```python
from build123d import *

# Parameters (mm, degrees)
BOSS_EXTRUDE1_DEPTH = 150
SKETCH2_R           = 1.500003704
SKETCH2_R_2         = 1.500002005
SKETCH2_R_3         = 1.500336032
SKETCH2_R_4         = 1.499979566
CUT_EXTRUDE1_DEPTH  = 5
SKETCH7_W           = 12.7
SKETCH7_H           = 16.8
CUT_EXTRUDE2_DEPTH  = 13
SKETCH8_W           = 16.8
SKETCH8_H           = 12.7
CUT_EXTRUDE3_DEPTH  = 13
SKETCH9_W           = 12.7
SKETCH9_H           = 16.8
CUT_EXTRUDE4_DEPTH  = 13
SKETCH10_W          = 18.7
SKETCH10_H          = 22.8
CUT_EXTRUDE5_DEPTH  = 2
FILLET1_R           = 2
SKETCH12_W          = 22.8
SKETCH12_H          = 18.7
CUT_EXTRUDE6_DEPTH  = 2
FILLET2_R           = 2
SKETCH13_W          = 18.7
SKETCH13_H          = 22.8
CUT_EXTRUDE7_DEPTH  = 2
FILLET3_R           = 2


with BuildPart() as part:
    # Sketch1 → Boss-Extrude1 (new body)
    with BuildSketch(Plane.XY):
        with BuildLine():
            Line((10.572650429, 43.57995567), (10.572650429, -28.420041122))
            ThreePointArc((10.572650429, -28.420041122), (11.744224426, -31.248470954), (14.572654257, -32.420044951))
            Line((14.572654257, -32.420044951), (86.572574673, -32.420044951))
            ThreePointArc((86.572574673, -32.420044951), (89.401092734, -31.248434409), (90.572703276, -28.419916348))
            Line((90.572703276, -28.419916348), (90.572703276, 43.558936727))
            ThreePointArc((90.572703276, 43.558936727), (89.3949748, 46.402224786), (86.551686742, 47.579953261))
            Line((86.551686742, 47.579953261), (14.57264802, 47.579953261))
            ThreePointArc((14.57264802, 47.579953261), (11.744222599, 46.408381091), (10.572650429, 43.57995567))
        make_face()
        with BuildLine():
            Line((16.572650429, 37.579953261), (16.572650429, -22.420044951))
            ThreePointArc((16.572650429, -22.420044951), (17.744223304, -25.248472075), (20.572650429, -26.420044951))
            Line((20.572650429, -26.420044951), (80.572648641, -26.420044951))
            ThreePointArc((80.572648641, -26.420044951), (83.401075766, -25.248472075), (84.572648641, -22.420044951))
            Line((84.572648641, -22.420044951), (84.572648641, 37.579953261))
            ThreePointArc((84.572648641, 37.579953261), (83.401075766, 40.408380386), (80.572648641, 41.579953261))
            Line((80.572648641, 41.579953261), (20.572650429, 41.579953261))
            ThreePointArc((20.572650429, 41.579953261), (17.744223304, 40.408380386), (16.572650429, 37.579953261))
        make_face(mode=Mode.SUBTRACT)
    extrude(amount=BOSS_EXTRUDE1_DEPTH)

    # Sketch2 → Cut-Extrude1 (cut)
    with BuildSketch(Plane.XY.offset(150)):
        with Locations((14.572654257, -28.420041122)):
            Circle(SKETCH2_R)
        with Locations((14.57264802, 43.57995567)):
            Circle(SKETCH2_R_2)
        with Locations((86.551686742, 43.558936727)):
            Circle(SKETCH2_R_3)
        with Locations((86.572574673, -28.419916348)):
            Circle(SKETCH2_R_4)
    cut_extrude1 = extrude(amount=-CUT_EXTRUDE1_DEPTH, mode=Mode.SUBTRACT)

    # Mirror1: Cut-Extrude1 across plane
    add(cut_extrude1.mirror(Plane(origin=(0, 0, 75), x_dir=(1, 0, 0), z_dir=(0, 0, -1))), mode=Mode.SUBTRACT)

    # Sketch7 → Cut-Extrude2 (cut)
    with BuildSketch(Plane(origin=(0, 47.579953261, 0), x_dir=(1, 0, 0), z_dir=(0, 1, 0))):
        with Locations((50.562167381, -40)):
            Rectangle(SKETCH7_W, SKETCH7_H)
    extrude(amount=-CUT_EXTRUDE2_DEPTH, mode=Mode.SUBTRACT)

    # Sketch8 → Cut-Extrude3 (cut)
    with BuildSketch(Plane(origin=(90.572703276, 0, 0), x_dir=(0, 0, -1), z_dir=(1, 0, 0))):
        with Locations((-80, 7.569510189)):
            Rectangle(SKETCH8_W, SKETCH8_H)
    extrude(amount=-CUT_EXTRUDE3_DEPTH, mode=Mode.SUBTRACT)

    # Sketch9 → Cut-Extrude4 (cut)
    with BuildSketch(Plane.XZ.offset(32.420044951)):
        with Locations((50.572614465, 120)):
            Rectangle(SKETCH9_W, SKETCH9_H)
    extrude(amount=-CUT_EXTRUDE4_DEPTH, mode=Mode.SUBTRACT)

    # Sketch10 → Cut-Extrude5 (cut)
    with BuildSketch(Plane(origin=(0, 47.579953261, 0), x_dir=(1, 0, 0), z_dir=(0, 1, 0))):
        with Locations((50.562167381, -40)):
            Rectangle(SKETCH10_W, SKETCH10_H)
    extrude(amount=-CUT_EXTRUDE5_DEPTH, mode=Mode.SUBTRACT)

    # Fillet1
    fillet1_edges = [part.edges().sort_by_distance(p)[0] for p in [
        (59.912167381, 46.579953261, 28.6),
        (59.912167381, 46.579953261, 51.4),
        (41.212167381, 46.579953261, 51.4),
        (41.212167381, 46.579953261, 28.6),
    ]]
    fillet(fillet1_edges, radius=FILLET1_R)

    # Sketch12 → Cut-Extrude6 (cut)
    with BuildSketch(Plane(origin=(90.572703276, 0, 0), x_dir=(0, 0, -1), z_dir=(1, 0, 0))):
        with Locations((-80, 7.569510189)):
            Rectangle(SKETCH12_W, SKETCH12_H)
    extrude(amount=-CUT_EXTRUDE6_DEPTH, mode=Mode.SUBTRACT)

    # Fillet2
    fillet2_edges = [part.edges().sort_by_distance(p)[0] for p in [
        (89.572703276, 16.919510189, 91.4),
        (89.572703276, 16.919510189, 68.6),
        (89.572703276, -1.780489811, 68.6),
        (89.572703276, -1.780489811, 91.4),
    ]]
    fillet(fillet2_edges, radius=FILLET2_R)

    # Sketch13 → Cut-Extrude7 (cut)
    with BuildSketch(Plane.XZ.offset(32.420044951)):
        with Locations((50.572614465, 120)):
            Rectangle(SKETCH13_W, SKETCH13_H)
    extrude(amount=-CUT_EXTRUDE7_DEPTH, mode=Mode.SUBTRACT)

    # Fillet3
    fillet3_edges = [part.edges().sort_by_distance(p)[0] for p in [
        (41.222614465, -31.420044951, 108.6),
        (41.222614465, -31.420044951, 131.4),
        (59.922614465, -31.420044951, 131.4),
        (59.922614465, -31.420044951, 108.6),
    ]]
    fillet(fillet3_edges, radius=FILLET3_R)


solid = part.part
```
Geometry check sheet. Reference: the model listing, model coordinates, mm. A direction names the side the tool comes from. Give positions to 0.01 mm unless a question says otherwise; leave off trailing zeros. Loops run counter-clockwise (first coordinate to the right, second up) from the corner with the lowest first, then second, coordinate; pieces in that order, holes last. Notation, with made-up numbers: (62.25, -15) - (104.25, -15) arc R18 ccw to (104.25, 6) - close; hole circle Ø10 at (21.25, -22). An arc over 180 degrees is marked (long way). Use CSV: the item, a comma, the result in double quotes. Start each with the question number.
Q1. Section check D-D, the plane z = 124.5. Record the cut outline in (x, y).
Q2. Section check A-A, the plane x = 66. Record the cut outline in (y, z), and give its area (3 significant figures).
Q3. Section check B-B, the plane z = 106. Record the cut outline in (x, y).
Q4. Access from +Z, -Z, +X, -X, +Y, -Y to the whole of each face (thin tool, end or side, straight path). Record for faces 1 (the face through (87, 44, 145)), 2 (the face through (17.713, -25.217, 73.95)), 3 (the face through (15, -28, 5)), 4 (the face through (50, -28, 111.6)), 5 (the face through (50, 44, 31.6)).
Q5. Release check for a two-part mould opening along X. For faces 6 (the face through (88.573, 16, 80)), 7 (the face through (11.775, 46.439, 73.95)), 8 (the face through (56.912, 44, 40)) record: +X half, -X half, draft (parallel to the pull), parting line (faces both ways), or undercut.
Q6. Section check C-C, the plane y = -4.5. Record the cut outline in (x, z), and give its area (3 significant figures).
Q7. Scan lines: probe 1 along X at (y, z) = (-0.5, 92); probe 2 along Y at (x, z) = (31, 67.5); probe 3 along Y at (x, z) = (56, 127). Record each from-to range of solid material in increasing order. Write a range as from..to.
Q8. Go/stop test with flat-tipped pins: pin 1 Ø1.8 at (x, y) = (14.57, -28.42) entering from +Z; pin 2 Ø1.8 at (x, y) = (86.55, 43.56) entering from -Z. Record where each tip stops, or that it passes through.
Findings below:
1,outline,"(10.57, -28.42) arc R4 ccw to (14.57, -32.42) - (41.22, -32.42) - (41.22, -30.42) - (44.22, -30.42) - (44.22, -26.42) - (20.57, -26.42) arc R4 cw to (16.57, -22.42) - (16.57, 37.58) arc R4 cw to (20.57, 41.58) - (80.57, 41.58) arc R4 cw to (84.57, 37.58) - (84.57, -22.42) arc R4 cw to (80.57, -26.42) - (56.92, -26.42) - (56.92, -30.42) - (59.92, -30.42) - (59.92, -32.42) - (86.57, -32.42) arc R4 ccw to (90.57, -28.42) - (90.57, 43.56) arc R4.02 ccw to (86.55, 47.58) - (14.57, 47.58) arc R4 ccw to (10.57, 43.58) - close"
2,outline,"(-32.42, 0) - (-26.42, 0) - (-26.42, 150) - (-32.42, 150) - close; (41.58, 0) - (47.58, 0) - (47.58, 150) - (41.58, 150) - close"
2,area,"1,800 mm^2"
3,outline,"(10.57, -28.42) arc R4 ccw to (14.57, -32.42) - (86.57, -32.42) arc R4 ccw to (90.57, -28.42) - (90.57, 43.56) arc R4.02 ccw to (86.55, 47.58) - (14.57, 47.58) arc R4 ccw to (10.57, 43.58) - close; hole (16.57, -22.42) arc R4 ccw to (20.57, -26.42) - (80.57, -26.42) arc R4 ccw to (84.57, -22.42) - (84.57, 37.58) arc R4 ccw to (80.57, 41.58) - (20.57, 41.58) arc R4 ccw to (16.57, 37.58) - close"
4,face 1,"+Z"
4,face 2,"+Z, -Z"
4,face 3,"-Z"
4,face 4,"-Y"
4,face 5,"+Y"
5,face 6,"+X half"
5,face 7,"-X half"
5,face 8,"undercut"
6,outline,"(10.57, 0) - (16.57, 0) - (16.57, 150) - (10.57, 150) - close; (84.57, 0) - (90.57, 0) - (90.57, 150) - (84.57, 150) - close"
6,area,"1,800 mm^2"
7,probe 1,"x = 10.57..16.57, 84.57..90.57"
7,probe 2,"y = -32.42..-26.42, 41.58..47.58"
7,probe 3,"y = 41.58..47.58"
8,pin 1,"stops at z = 145"
8,pin 2,"stops at z = 5"
